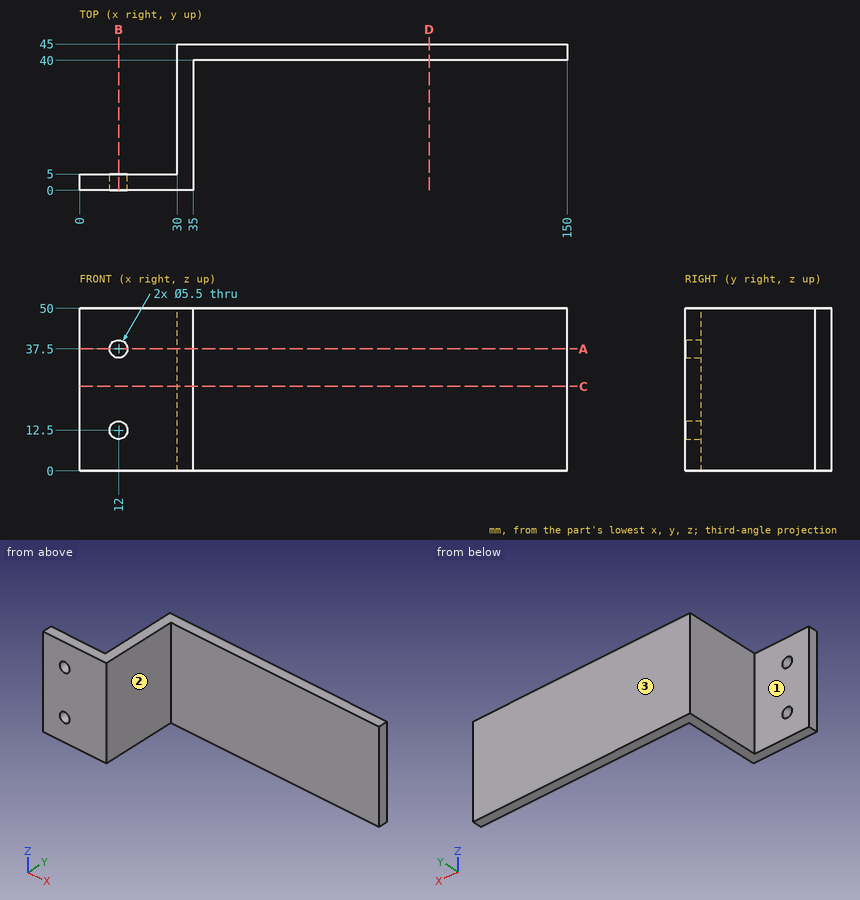
Job drawing, mm, ordinate dimensions from the low corner. One solid piece. A direction names the side the tool comes from. Round coordinates to 2 decimals unless told otherwise and drop trailing zeros. Loops run counter-clockwise (first coordinate to the right, second up) from the corner with the lowest first, then second, coordinate; pieces in that order, holes last. Notation, with made-up numbers: (14.25, 8) -> (67.25, 8) arc R17 cw to (67.25, 29) -> close; hole circle Ø5 at (55.5, -25.75). An arc over 180 degrees is marked (long way). Use a Markdown table: item, result.
1) Cut at A-A, the plane z = 37.5. List the corners of the cut face in (x, y).
The answers:
| item | result |
|---|---|
| outline | (0, 0) -> (9.25, 0) -> (9.25, 5) -> (0, 5) -> close; (14.75, 0) -> (35, 0) -> (35, 40) -> (150, 40) -> (150, 45) -> (30, 45) -> (30, 5) -> (14.75, 5) -> close |
2) Tool access for the marked faces 1, 2 and 3: list every direction of +Z, -Z, +X, -X, +Y, -Y with a clear straight run to the whole face (end or side of a thin tool).
The answers:
| item | result |
|---|---|
| face 1 | +Z, -Z, -X, +Y |
| face 2 | +Z, -Z, +X, -Y |
| face 3 | +Z, -Z, +X, -X, +Y |
3) Cut at D-D, the plane x = 107.5. List the corners of the cut face in (y, z).
The answers:
| item | result |
|---|---|
| outline | (40, 0) -> (45, 0) -> (45, 50) -> (40, 50) -> close |
4) Probe line 1 (X direction, y = 1.75, z = 37.5); line 2 (X direction, y = 9.5, z = 14); line 3 (Y direction, x = 76.5, z = 20.5). List the from-to ranges inside material, lowest first. Write a range as [from, to].
The answers:
| item | result |
|---|---|
| line 1 | x = [0, 9.25], [14.75, 35] |
| line 2 | x = [30, 35] |
| line 3 | y = [40, 45] |
5) Drop flat-ended pins along their axis: pin 1 Ø12 at (y, z) = (11, 27.5) entering from +X; pin 2 Ø15 at (x, z) = (19.5, 23.5) entering from +Y; pin 3 Ø8 at (x, z) = (111.5, 19) entering from -Y. Give the stop position or say it passes through.
The answers:
| item | result |
|---|---|
| pin 1 | stops at x = 35 |
| pin 2 | stops at y = 5 |
| pin 3 | stops at y = 40 |
6) Cut at B-B, the plane x = 12. List the corners of the cut face in (y, z).
The answers:
| item | result |
|---|---|
| outline | (0, 0) -> (5, 0) -> (5, 9.75) -> (0, 9.75) -> close; (0, 15.25) -> (5, 15.25) -> (5, 34.75) -> (0, 34.75) -> close; (0, 40.25) -> (5, 40.25) -> (5, 50) -> (0, 50) -> close |
7) Cut at C-C, the plane z = 26. List the corners of the cut face in (x, y).
The answers:
| item | result |
|---|---|
| outline | (0, 0) -> (35, 0) -> (35, 40) -> (150, 40) -> (150, 45) -> (30, 45) -> (30, 5) -> (0, 5) -> close |
